Design review of the part built by this model. Coordinates are the model's own, in mm. Coordinates: 2 decimals unless noted, no trailing zeros. Write each loop counter-clockwise with the first axis right and the second up, starting at its lowest first coordinate (ties: lowest second). Pieces come first, ordered by that corner, then holes. Notation, with made-up numbers: (-18, 47.5) - (38, 47.5) arc R29 ccw to (38, 75.5) - close; hole circle Ø7 at (8.5, -31.5). An arc over 180 degrees is marked (long way). Answer as a JSON object with one key per item and string values.
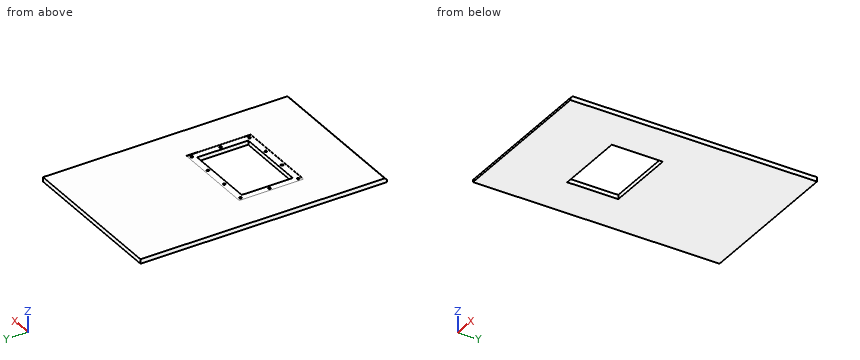
```python
from build123d import *

# Parameters (mm, degrees)
SKETCH1_W                     = 700
SKETCH1_H                     = 1110
SKETCH1_W_2                   = 320
SKETCH1_H_2                   = 230
BOSS_EXTRUDE1_DEPTH           = 20
SKETCH2_W                     = 380
SKETCH2_H                     = 290
CUT_EXTRUDE1_DEPTH            = 1
F_1_2_13_THREADED_HOLE1_D     = 10.71626
F_1_2_13_THREADED_HOLE1_DEPTH = 14
F_1_2_13_THREADED_HOLE1_TIP   = 3.219489309
CHAMFER1_SIZE                 = 10


with BuildPart() as part:
    # Sketch1 → Boss-Extrude1 (new body)
    with BuildSketch(Plane.XY):
        with Locations((350, 555)):
            Rectangle(SKETCH1_W, SKETCH1_H)
        with Locations((350, 420)):
            Rectangle(SKETCH1_W_2, SKETCH1_H_2, mode=Mode.SUBTRACT)
    extrude(amount=BOSS_EXTRUDE1_DEPTH)

    # Sketch2 → Cut-Extrude1 (cut)
    with BuildSketch(Plane.XY.offset(20)):
        with Locations((350, 420)):
            Rectangle(SKETCH2_W, SKETCH2_H)
    extrude(amount=-CUT_EXTRUDE1_DEPTH, mode=Mode.SUBTRACT)

    # 1/2-13 Threaded hole1
    with Locations(Plane(origin=(175, 550, 19), x_dir=(1, 0, 0), z_dir=(0, 0, 1))):
        with Locations((0, 0), (116.5, 0), (233.5, 0), (350, 0), (350, -130), (350, -260), (233.5, -260), (116.5, -260), (0, -260), (0, -130)):
            Hole(F_1_2_13_THREADED_HOLE1_D / 2, depth=F_1_2_13_THREADED_HOLE1_DEPTH)
            with Locations((0, 0, -(F_1_2_13_THREADED_HOLE1_DEPTH + F_1_2_13_THREADED_HOLE1_TIP / 2))):  # 118° drill point
                Cone(0, F_1_2_13_THREADED_HOLE1_D / 2, F_1_2_13_THREADED_HOLE1_TIP, mode=Mode.SUBTRACT)

    # Chamfer1
    chamfer1_edges = [part.edges().sort_by_distance(p)[0] for p in [
        (350, 0, 20),
    ]]
    chamfer(chamfer1_edges, length=CHAMFER1_SIZE)


solid = part.part
```
(1) To check wall thickness, follow line 1 (X direction, y = 550, z = 14.5); line 2 (Y direction, x = 175, z = 10.25); line 3 (Y direction, x = 175, z = 9.75). State the ranges of each line that lie inside material, in increasing order. Write a range as from..to.
Solved:
{"line 1": "x = 0..169.64, 180.36..286.14, 296.86..403.14, 413.86..519.64, 530.36..700", "line 2": "y = 0.25..284.64, 295.36..414.64, 425.36..544.64, 555.36..1110", "line 3": "y = 0..284.64, 295.36..414.64, 425.36..544.64, 555.36..1110"}
(2) For pin 1 (12.5 mm diameter, centred on x = 525, y = 550, fed in from -Z); pin 2 (8.5 mm diameter, centred on x = 408.5, y = 550, fed in from +Z); pin 3 (0.8 mm diameter, centred on x = 285, z = 19.5, fed in from -Y); pin 4 (6.5 mm diameter, centred on x = 291.5, y = 290, fed in from +Z), all flat-tipped, find the tip position at first contact; note any pin that passes through.
Solved:
{"pin 1": "stops at z = 0", "pin 2": "stops at z = 4.33", "pin 3": "stops at y = 9.1", "pin 4": "stops at z = 3.73"}
(3) Take a section at A-A, the plane y = 469.5. Write out the cut boundary in (x, z).
Solved:
{"outline": "(0, 0) - (190, 0) - (190, 19) - (160, 19) - (160, 20) - (0, 20) - close; (510, 0) - (700, 0) - (700, 20) - (540, 20) - (540, 19) - (510, 19) - close"}
